Could you check a few things on this model? Use its own coordinates, in mm. Face numbers are marked on the shaded views. A direction names the side the tool comes from. Coordinates: 2 decimals unless noted, no trailing zeros. Order: outer loops, then holes, each group sorted by start corner. A loop starts at its lowest first (then second) coordinate and runs counter-clockwise, first axis right, second up. Notation, with made-up numbers: (16.25, 52) -> (36.25, 52) arc R20 ccw to (36.25, 74) -> close; hole circle Ø1 at (15, -32). An arc over 180 degrees is marked (long way). Put each result on its own line as item: value. Start each with the question number.
Q1. Will these pins go through, and if not, where does the flat tip stop? pin 1 (5 mm diameter, centred on x = 8, z = 3.5, fed in from -Y); pin 2 (3 mm diameter, centred on y = -2, z = 5.5, fed in from +X).
Q2. If we section it at A-A (z = 3.75): Please give me the cut outline in (x, y), and give its area (3 significant figures).
Q3. If we section it at B-B (x = 12): Please give me the cut outline in (y, z).
Q4. If we section it at C-C (y = 6.5): Please give me the cut outline in (x, z).
Q5. Please list where these lines run through material, in increasing order: line 1 along Y through (x, z) = (9, 9.25); line 2 along X through (y, z) = (7, 6.75).
Q6. For the marked faces 1, 2 and 3, which set-ups out of +Z, -Z, +X, -X, +Y, -Y let a thin tool reach every point of the face, with its end or its side?
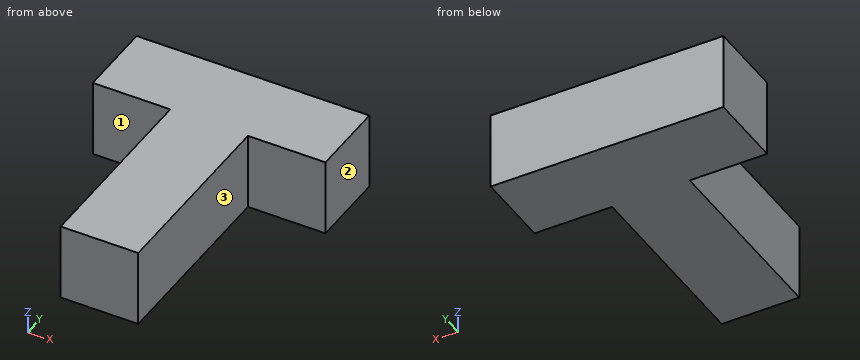
from build123d import *

# Parameters (mm, degrees)
SKETCH1_W           = 30
SKETCH1_H           = 35
BOSS_EXTRUDE1_DEPTH = 10
SKETCH2_W           = 10
SKETCH2_H           = 25
CUT_EXTRUDE1_DEPTH  = 26.124689053


with BuildPart() as part:
    # Sketch1 → Boss-Extrude1 (new body)
    with BuildSketch(Plane.XY):
        Rectangle(SKETCH1_W, SKETCH1_H)
    extrude(amount=BOSS_EXTRUDE1_DEPTH)

    # Sketch2 → Cut-Extrude1 (cut, through all)
    with BuildSketch(Plane.XY.offset(10)):
        with Locations((-10, -5)):
            Rectangle(SKETCH2_W, SKETCH2_H)
        with Locations((10, -5)):
            Rectangle(SKETCH2_W, SKETCH2_H)
    extrude(amount=-CUT_EXTRUDE1_DEPTH, mode=Mode.SUBTRACT)


solid = part.part
The answers:
1. pin 1: y = 7.5
1. pin 2: x = 5
2. outline: (-15, 7.5) -> (-5, 7.5) -> (-5, -17.5) -> (5, -17.5) -> (5, 7.5) -> (15, 7.5) -> (15, 17.5) -> (-15, 17.5) -> close
2. area: 550 mm^2
3. outline: (7.5, 0) -> (17.5, 0) -> (17.5, 10) -> (7.5, 10) -> close
4. outline: (-5, 0) -> (5, 0) -> (5, 10) -> (-5, 10) -> close
5. line 1: 7.5 to 17.5
5. line 2: -5 to 5
6. face 1: +Z, -Z, -X, -Y
6. face 2: +Z, -Z, +X, +Y, -Y
6. face 3: +Z, -Z, +X, -Y
